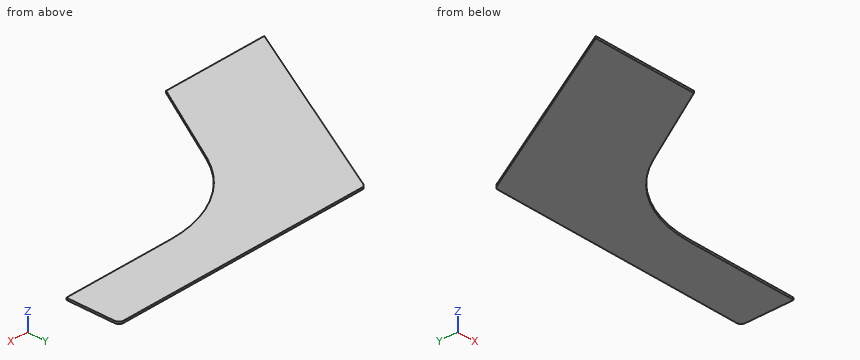
```python
from build123d import *

# Parameters (mm, degrees)
BOSS_EXTRUDE1_DEPTH = 1.5


with BuildPart() as part:
    # Sketch1 → Boss-Extrude1 (new body)
    with BuildSketch(Plane.XY):
        with BuildLine():
            Line((0, 0), (79.011764706, 148.147058824))
            ThreePointArc((79.011764706, 148.147058824), (80.299264856, 149.50122524), (82.1, 150))
            Line((82.1, 150), (276.5, 150))
            ThreePointArc((276.5, 150), (278.974873734, 148.974873734), (280, 146.5))
            Line((280, 146.5), (280, 110))
            Line((280, 110), (195, 110))
            ThreePointArc((195, 110), (149.787439916, 97.819177653), (116.813238993, 64.573875793))
            Line((116.813238993, 64.573875793), (80, 0))
            Line((80, 0), (0, 0))
        make_face()
    extrude(amount=BOSS_EXTRUDE1_DEPTH)


solid = part.part
```
CAD build for the part. Positions are in the model's coordinates, mm. Give positions to 0.01 mm unless a question says otherwise; leave off trailing zeros. Order: outer loops, then holes, each group sorted by start corner. A loop starts at its lowest first (then second) coordinate and runs counter-clockwise, first axis right, second up. Notation, with made-up numbers: M 87.5,62 L 99.5,62 A21 ccw 99.5,94 Z; hole C 62.25,75.25 d1. An arc over 180 degrees is marked long. Put each result on its own line as item: value. Start each with the question number.
(1) Drill centre lines: line 1 along Y through (x, z) = (235, 1.25); line 2 along Y through (x, z) = (181.5, 0.55); line 3 along X through (y, z) = (89, 0.95). Where is each one in solid material? Low to high.
(2) Saw through at A-A, the plane z = 0.55. Write the cut outline in (x, y).
(3) Saw through at B-B, the plane x = 68. Write the cut outline in (y, z), then the cut area to 3 significant figures.
(4) Saw through at C-C, the plane y = 16. Write the cut outline in (x, z).
Check result:
1. line 1: y = 110 to 150
1. line 2: y = 108.98 to 150
1. line 3: x = 47.47 to 137.22
2. outline: M 0,0 L 80,0 L 116.81,64.57 A90 cw 195,110 L 280,110 L 280,146.5 A3.5 ccw 276.5,150 L 82.1,150 A3.5 ccw 79.01,148.15 Z
3. outline: M 0,0 L 127.5,0 L 127.5,1.5 L 0,1.5 Z
3. area: 191 mm2
4. outline: M 8.53,0 L 89.12,0 L 89.12,1.5 L 8.53,1.5 Z
